Design review of the part built by this model. Coordinates are the model's own, in mm. Face numbers are marked on the shaded views. A direction names the side the tool comes from. Round coordinates to 2 decimals unless told otherwise and drop trailing zeros. Loops run counter-clockwise (first coordinate to the right, second up) from the corner with the lowest first, then second, coordinate; pieces in that order, holes last. Notation, with made-up numbers: (-5, -33) - (41, -33) arc R27 cw to (41, 4) - close; hole circle Ø6 at (69.25, -32.5). An arc over 180 degrees is marked (long way). Use one line per item in the form item = value. Start each with the question number.
(1) Wall thickness on probe 1 along Y at (x, z) = (27.5, 96); probe 2 along X at (y, z) = (11, 127.5): over which ranges is each line inside the solid? List them lowest first. Write a range as [from, to].
(2) Machinability: for the marked faces 1 and 2, which of the approach directions +Z, -Z, +X, -X, +Y, -Y give a long, thin tool a straight path to every point of the face, cutting with its end or side? Answer none if there is none.
(3) We need section D-D, the plane x = 23.25. Write out the cut boundary in (y, z), then the cut area to 3 significant figures.
(4) We need section C-C, the plane z = 117. Write out the cut boundary in (x, y), then the cut area to 3 significant figures.
(5) We need section A-A, the plane z = 77.5. Write out the cut boundary in (x, y).
(6) We need section B-B, the plane y = 25. Write out the cut boundary in (x, z), then the cut area to 4 significant figures.
(7) For pin 1 (5 mm diameter, centred on x = 4, z = 31, fed in from +Y); pin 2 (15.5 mm diameter, centred on y = 11.5, z = 72.5, fed in from -X); pin 3 (0.8 mm diameter, centred on y = 1, z = 62, fed in from +X), all flat-tipped, find the tip position at first contact; note any pin that passes through.
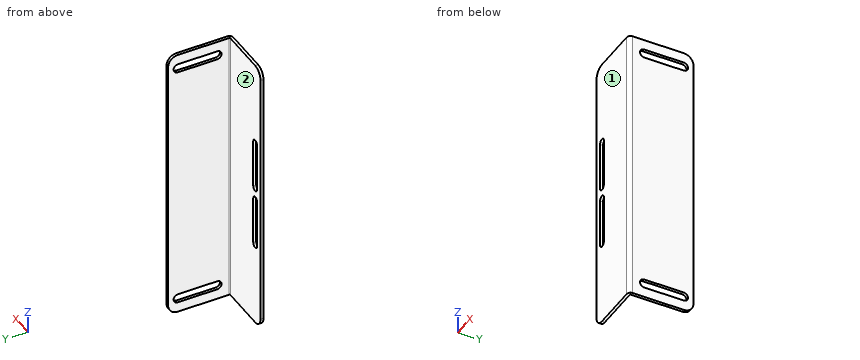
from build123d import *

# Parameters (mm, degrees)
SKETCH_1_W          = 30
SKETCH_1_H          = 33
EXTRUDE_1_DEPTH     = 144
SHELL_1_T           = -1.5
FILLET_1_R          = 5
FILLET_2_R          = 0.5
FILLET_3_R          = 2
CUT_EXTRUDE_1_DEPTH = 198.864221121
CUT_EXTRUDE_2_REACH = 152.748
SKETCH_3_R          = 1.75
CUT_EXTRUDE_3_DEPTH = 1.5


with BuildPart() as part:
    # 草图1 → 凸台-拉伸1 (new body)
    with BuildSketch(Plane.XY):
        with Locations((15, 16.5)):
            Rectangle(SKETCH_1_W, SKETCH_1_H)
    extrude(amount=EXTRUDE_1_DEPTH)

    # 抽壳1
    shell_1_openings = [part.faces().sort_by_distance(p)[0] for p in [
        (15, 16.5, 144),
        (15, 16.5, 0),
        (15, 33, 72),
        (0, 16.5, 72),
    ]]
    offset(amount=SHELL_1_T, openings=shell_1_openings, kind=Kind.INTERSECTION)

    # 圆角1
    fillet_1_edges = [part.edges().sort_by_distance(p)[0] for p in [
        (29.25, 33, 144),
        (0, 0.75, 144),
        (29.25, 33, 0),
        (0, 0.75, 0),
    ]]
    fillet(fillet_1_edges, radius=FILLET_1_R)

    # 圆角2
    fillet_2_edges = [part.edges().sort_by_distance(p)[0] for p in [
        (28.5, 1.5, 72),
    ]]
    fillet(fillet_2_edges, radius=FILLET_2_R)

    # 圆角3
    fillet_3_edges = [part.edges().sort_by_distance(p)[0] for p in [
        (30, 0, 72),
    ]]
    fillet(fillet_3_edges, radius=FILLET_3_R)

    # 草图2 → 切除-拉伸1 (cut, through all)
    with BuildSketch(Plane(origin=(28.5, 0, -49), x_dir=(0, 0, 1), z_dir=(-1, 0, 0))):
        with BuildLine():
            Line((54.25, 8), (54.25, 28))
            ThreePointArc((54.25, 28), (56.5, 30.25), (58.75, 28))
            Line((58.75, 28), (58.75, 8))
            ThreePointArc((58.75, 8), (56.5, 5.75), (54.25, 8))
        make_face()
        with BuildLine():
            Line((187.75, 28), (187.75, 8))
            ThreePointArc((187.75, 8), (185.5, 5.75), (183.25, 8))
            Line((183.25, 8), (183.25, 28))
            ThreePointArc((183.25, 28), (185.5, 30.25), (187.75, 28))
        make_face()
    extrude(amount=-CUT_EXTRUDE_1_DEPTH, mode=Mode.SUBTRACT)

    # 草图3 → 切除-拉伸2 (cut, up to next)
    with BuildSketch(Plane(origin=(0, 0, 0), x_dir=(1, 0, 0), z_dir=(0, 1, 0)), mode=Mode.PRIVATE) as cut_extrude_2_sk1:
        with Locations(Location((5, -87.875, 0), (0, 0, 270))):
            Circle(SKETCH_3_R)
    cut_extrude_2_tool1 = extrude(cut_extrude_2_sk1.sketch, amount=CUT_EXTRUDE_2_REACH, mode=Mode.PRIVATE) & part.part
    # 草图3 → 切除-拉伸2 (cut, up to next)
    with BuildSketch(Plane(origin=(0, 0, 0), x_dir=(1, 0, 0), z_dir=(0, 1, 0)), mode=Mode.PRIVATE) as cut_extrude_2_sk2:
        with Locations(Location((5, -56.125, 0), (0, 0, 270))):
            Circle(SKETCH_3_R)
    cut_extrude_2_tool2 = extrude(cut_extrude_2_sk2.sketch, amount=CUT_EXTRUDE_2_REACH, mode=Mode.PRIVATE) & part.part
    add(cut_extrude_2_tool1.solids().sort_by_distance((5, 0, 87.875))[0], mode=Mode.SUBTRACT)
    add(cut_extrude_2_tool2.solids().sort_by_distance((5, 0, 56.125))[0], mode=Mode.SUBTRACT)

    # 草图4 → 切除-拉伸3 (cut)
    with BuildSketch(Plane(origin=(0, 0, 0), x_dir=(1, 0, 0), z_dir=(0, 1, 0))):
        with BuildLine():
            Line((3.25, -100.375), (3.25, -75.375))
            ThreePointArc((3.25, -75.375), (5, -73.625), (6.75, -75.375))
            Line((6.75, -75.375), (6.75, -100.375))
            ThreePointArc((6.75, -100.375), (5, -102.125), (3.25, -100.375))
        make_face()
        with BuildLine():
            Line((3.25, -68.625), (3.25, -43.625))
            ThreePointArc((3.25, -43.625), (5, -41.875), (6.75, -43.625))
            Line((6.75, -43.625), (6.75, -68.625))
            ThreePointArc((6.75, -68.625), (5, -70.375), (3.25, -68.625))
        make_face()
    extrude(amount=CUT_EXTRUDE_3_DEPTH, mode=Mode.SUBTRACT)


solid = part.part
Data:
q1.probe_1 = [0, 1.5]
q1.probe_2 = [28.5, 30]
q2.face_1 = +Z, -Z, +X, -X, -Y
q2.face_2 = +Z, -Z, -X, +Y
q3.outline = (0, 0) - (1.5, 0) - (1.5, 144) - (0, 144) - close
q3.area = 216 mm^2
q4.outline = (0, 0) - (28, 0) arc R2 ccw to (30, 2) - (30, 33) - (28.5, 33) - (28.5, 2) arc R0.5 cw to (28, 1.5) - (0, 1.5) - close
q4.area = 91.4 mm^2
q5.outline = (0, 0) - (3.25, 0) - (3.25, 1.5) - (0, 1.5) - close; (6.75, 0) - (28, 0) arc R2 ccw to (30, 2) - (30, 33) - (28.5, 33) - (28.5, 2) arc R0.5 cw to (28, 1.5) - (6.75, 1.5) - close
q6.outline = (28.5, 0) - (30, 0) - (30, 5.25) - (28.5, 5.25) - close; (28.5, 9.75) - (30, 9.75) - (30, 134.25) - (28.5, 134.25) - close; (28.5, 138.75) - (30, 138.75) - (30, 144) - (28.5, 144) - close
q6.area = 202.5 mm^2
q7.pin_1 = 1.5
q7.pin_2 = 28.5
q7.pin_3 = 29.91
